from build123d import *

# Parameters (mm, degrees)
SKETCH_1_W                = 42
SKETCH_1_H                = 41
EXTRUDE_1_DEPTH           = 15
SKETCH_2_R                = 12.75
CUT_EXTRUDE_1_DEPTH       = 15
SKETCH_3_W                = 2
SKETCH_3_H                = 38
CUT_EXTRUDE_2_DEPTH       = 15
HOLE_WIZARD_M6_1_D        = 5
HOLE_WIZARD_M6_1_DEPTH    = 17
HOLE_WIZARD_M6_1_TIP      = 1.502151548
HOLE_WIZARD_7_0_7_1_D     = 7
HOLE_WIZARD_7_0_7_1_DEPTH = 20
HOLE_WIZARD_M6_2_D        = 5
CHAMFER_1_SIZE            = 0.5
CHAMFER_2_SIZE            = 0.5


with BuildPart() as part:
    # 草图1 → 凸台-拉伸1 (new body)
    with BuildSketch(Plane.XY):
        with Locations((21, 20.5)):
            Rectangle(SKETCH_1_W, SKETCH_1_H)
    extrude(amount=EXTRUDE_1_DEPTH)

    # 草图2 → 切除-拉伸1 (cut)
    with BuildSketch(Plane.XY.offset(15)):
        with Locations((21, 22.5)):
            Circle(SKETCH_2_R)
    extrude(amount=-CUT_EXTRUDE_1_DEPTH, mode=Mode.SUBTRACT)

    # 草图3 → 切除-拉伸2 (cut)
    with BuildSketch(Plane.XY.offset(15)):
        with Locations((21, 19)):
            Rectangle(SKETCH_3_W, SKETCH_3_H)
    extrude(amount=-CUT_EXTRUDE_2_DEPTH, mode=Mode.SUBTRACT)

    # M6 螺纹孔1
    with Locations(Plane(origin=(0, 41, 0), x_dir=(1, 0, 0), z_dir=(0, 1, 0))):
        with Locations((5, -7.5), (37, -7.5)):
            Hole(HOLE_WIZARD_M6_1_D / 2, depth=HOLE_WIZARD_M6_1_DEPTH)
            with Locations((0, 0, -(HOLE_WIZARD_M6_1_DEPTH + HOLE_WIZARD_M6_1_TIP / 2))):  # 118° drill point
                Cone(0, HOLE_WIZARD_M6_1_D / 2, HOLE_WIZARD_M6_1_TIP, mode=Mode.SUBTRACT)

    # Ø7.0 (7) 直径孔1
    with Locations(Plane.ZY):
        with Locations((7.5, 5)):
            Hole(HOLE_WIZARD_7_0_7_1_D / 2, depth=HOLE_WIZARD_7_0_7_1_DEPTH)

    # M6 螺纹孔2 (through all)
    with Locations(Plane.ZY.offset(-22)):
        with Locations((7.5, 5)):
            Hole(HOLE_WIZARD_M6_2_D / 2)

    # 倒角1
    chamfer_1_edges = [part.edges().sort_by_distance(p)[0] for p in [
        (33.75, 22.5, 0),
        (33.75, 22.5, 15),
    ]]
    chamfer(chamfer_1_edges, length=CHAMFER_1_SIZE)

    # 倒角2
    chamfer_2_edges = [part.edges().sort_by_distance(p)[0] for p in [
        (8.25, 22.5, 0),
        (8.25, 22.5, 15),
    ]]
    chamfer(chamfer_2_edges, length=CHAMFER_2_SIZE)


solid = part.part
For this review, take the finished solid that the model builds, in its own axes (mm). A direction names the side the tool comes from. Round coordinates to 2 decimals unless told otherwise and drop trailing zeros. Loops run counter-clockwise (first coordinate to the right, second up) from the corner with the lowest first, then second, coordinate; pieces in that order, holes last. Notation, with made-up numbers: (9.25, 54.25) - (14.25, 54.25) arc R30 cw to (14.25, 83.25) - close; hole circle Ø6 at (35.25, 72.5). An arc over 180 degrees is marked (long way). One line per item, written item: value. Start each with the question number.
Item 1: The part is to be moulded in two halves that separate along X. For faces 1 (the cylindrical face through (3.85, 32.38, 9.72)), 2 (the flat face through (42, 20, 7)), 3 (the flat face through (30, 12, 0)), say which applies: +X half, -X half, draft (parallel to the pull), parting line (faces both ways), or undercut.
Item 2: Take a section at C-C (z = 13). Give the boundary of the cut face in (x, y).
Item 3: Clearance check with flat-ended pins moving along their axes: pin 1 Ø4.5 at (x, z) = (37, 7.5) entering from +Y; pin 2 Ø1.6 at (x, z) = (21, 7) entering from -Y. State where each tip first meets the part, or that it passes through.
Item 4: Take a section at A-A (y = 37). Give the boundary of the cut face in (x, z).
Item 5: For L1, parallel to X at y = 2, z = 2; L2, parallel to Z at x = 37, y = 30; L3, parallel to X at y = 30.5, z = 9.25, list the stretches that pass through material, from the lowest coordinate up.
Item 6: For faces 4 (the flat face through (20, 37, 8)), 5 (the cylindrical face through (8.253, 22.766, 7.598)), 6 (the cylindrical face through (10, 5, 11)), list the 3-axis set-ups (+Z, -Z, +X, -X, +Y, -Y) from which the entire face can be reached by the end or side of a thin tool; tool diameter is ignored.
Item 7: Take a section at D-D (x = 9.5). State how many separate pieces and enclosed holes the cut face has, plus the area to 3 significant figures.
Item 8: Take a section at B-B (y = 5). Give the boundary of the cut face in (x, z), plus the area to 3 significant figures.
Answer below:
1. face 1: undercut
1. face 2: +X half
1. face 3: draft
2. outline: (0, 0) - (20, 0) - (20, 9.79) arc R12.75 cw to (20, 35.21) - (20, 38) - (22, 38) - (22, 35.21) arc R12.75 cw to (22, 9.79) - (22, 0) - (42, 0) - (42, 41) - (0, 41) - close
3. pin 1: stops at y = 23.85
3. pin 2: stops at y = 38
4. outline: (0, 0) - (20, 0) - (20, 15) - (0, 15) - close; (22, 0) - (42, 0) - (42, 15) - (22, 15) - close; hole circle Ø5 at (5, 7.5); hole circle Ø5 at (37, 7.5)
5. L1: x = 0 to 20, 22 to 42
5. L2: z = 0 to 5, 10 to 15
5. L3: x = 0 to 3.21, 6.79 to 11.07, 30.93 to 35.21, 38.79 to 42
6. face 4: +Z, -Z, -Y
6. face 5: +Z, -Z
6. face 6: -X
7. separate pieces: 2
7. enclosed holes: 1
7. area: 410 mm2
8. outline: (0, 0) - (20, 0) - (20, 4) - (0, 4) - close; (0, 11) - (20, 11) - (20, 15) - (0, 15) - close; (22, 0) - (42, 0) - (42, 5) - (22, 5) - close; (22, 10) - (42, 10) - (42, 15) - (22, 15) - close
8. area: 360 mm2
